```python
from build123d import *

# Parameters (mm, degrees)
SKETCH_1_W             = 46
SKETCH_1_H             = 55
EXTRUDE_1_DEPTH        = 5
HOLE_WIZARD_M27_1_0_D  = 24
FILLET_1_R             = 10
HOLE_WIZARD_M4_1_D     = 3.3
HOLE_WIZARD_M4_1_DEPTH = 11.5
HOLE_WIZARD_M4_1_TIP   = 0.991420021
CHAMFER_1_SIZE         = 2


with BuildPart() as part:
    # 草图1 → 凸台-拉伸1 (new, symmetric)
    with BuildSketch(Plane(origin=(0, 0, 0), x_dir=(1, 0, 0), z_dir=(0, 1, 0))):
        Rectangle(SKETCH_1_W, SKETCH_1_H)
    extrude(amount=EXTRUDE_1_DEPTH, both=True)

    # M27*1.0反牙 (through all)
    with Locations(Plane(origin=(0, 5, 0), x_dir=(1, 0, 0), z_dir=(0, 1, 0))):
        with Locations((0, -7.5)):
            Hole(HOLE_WIZARD_M27_1_0_D / 2)

    # 圆角1
    fillet_1_edges = [part.edges().sort_by_distance(p)[0] for p in [
        (23, 0, 27.5),
        (-23, 0, 27.5),
    ]]
    fillet(fillet_1_edges, radius=FILLET_1_R)

    # M4 螺纹孔1
    with Locations(Plane(origin=(0, 0, -27.5), x_dir=(-1, 0, 0), z_dir=(0, 0, -1))):
        with Locations((-15, 0), (15, 0)):
            Hole(HOLE_WIZARD_M4_1_D / 2, depth=HOLE_WIZARD_M4_1_DEPTH)
            with Locations((0, 0, -(HOLE_WIZARD_M4_1_DEPTH + HOLE_WIZARD_M4_1_TIP / 2))):  # 118° drill point
                Cone(0, HOLE_WIZARD_M4_1_D / 2, HOLE_WIZARD_M4_1_TIP, mode=Mode.SUBTRACT)

    # 倒角1
    chamfer_1_edges = [part.edges().sort_by_distance(p)[0] for p in [
        (-23, 0, -27.5),
        (23, 0, -27.5),
    ]]
    chamfer(chamfer_1_edges, length=CHAMFER_1_SIZE)


solid = part.part
```
CAD build for the part. Positions are in the model's coordinates, mm. A direction names the side the tool comes from. Coordinates: 2 decimals unless noted, no trailing zeros. Write each loop counter-clockwise with the first axis right and the second up, starting at its lowest first coordinate (ties: lowest second). Pieces come first, ordered by that corner, then holes.
(1) Flat gauge pins, fed straight in: pin 1 (8 mm diameter, centred on x = -3.5, z = -3, fed in from +Y); pin 2 (2.5 mm diameter, centred on x = 15, y = 0, fed in from +Z); pin 3 (14.5 mm diameter, centred on x = 0, z = 7.5, fed in from -Y). Where does each tip first touch, or does it go through?
(2) Drill centre lines: probe 1 along X at (y, z) = (0, -18.5); probe 2 along Y at (x, z) = (15, -19.75); probe 3 along Z at (x, y) = (-6.5, 0). Where is each one in solid material? Low to high.
(3) Cut at D-D, the plane z = -23. List the corners of the cut face in (x, y), and give its area (3 significant figures).
(4) Cut at A-A, the plane x = 11. List the corners of the cut face in (y, z).
(5) 3-axis set-ups, long thin cutter, end or side, ignore diameter. For faces 4 (the face through (0, -5, -6)), 5 (the face through (16.574, 0.496, -21.67)): which of +Z, -Z, +X, -X, +Y, -Y reach the whole face in a straight line?
(6) Cut at C-C, the plane y = -3.5. List the corners of the cut face in (x, z).
(7) Cut at B-B, the plane z = 1. List the corners of the cut face in (x, y).
(8) Two-plate mould, pull along X, no slides. Class faces 1 (the face through (-13.476, -0.632, -21.67)), 2 (the face through (-23, 0, -4)), 3 (the face through (19.99, 0.07, 24.65)): +X half, -X half, draft (parallel to the pull), parting line (faces both ways), or undercut.
Geometry says:
1. pin 1: stops at y = 5
1. pin 2: stops at z = 27.47
1. pin 3: passes through
2. probe 1: x = -23 to -16.65, -13.35 to 13.35, 16.65 to 23
2. probe 2: y = -5 to -1.65, 1.65 to 5
2. probe 3: z = -27.5 to -2.59, 17.59 to 27.5
3. outline: (-23, -5) - (23, -5) - (23, 5) - (-23, 5) - close; hole circle Ø3.3 at (-15, 0); hole circle Ø3.3 at (15, 0)
3. area: 443 mm2
4. outline: (-5, -27.5) - (5, -27.5) - (5, 2.7) - (-5, 2.7) - close; (-5, 12.3) - (5, 12.3) - (5, 27.5) - (-5, 27.5) - close
5. face 4: +Z, -Z, +X, -X, -Y
5. face 5: -Z
6. outline: (-23, -25.5) - (-21, -27.5) - (21, -27.5) - (23, -25.5) - (23, 17.5) arc R10 ccw to (13, 27.5) - (-13, 27.5) arc R10 ccw to (-23, 17.5) - close; hole circle Ø24 at (0, 7.5)
7. outline: (-23, -5) - (-10.09, -5) - (-10.09, 5) - (-23, 5) - close; (10.09, -5) - (23, -5) - (23, 5) - (10.09, 5) - close
8. face 1: undercut
8. face 2: -X half
8. face 3: +X half
